Part model, mm, in its own coordinate system. Round coordinates to 2 decimals unless told otherwise and drop trailing zeros. Order: outer loops, then holes, each group sorted by start corner. A loop starts at its lowest first (then second) coordinate and runs counter-clockwise, first axis right, second up. Notation, with made-up numbers: (-7.75, -11) - (18.25, -11) arc R20 ccw to (18.25, 7) - close; hole circle Ø9 at (-30.75, -22.5). An arc over 180 degrees is marked (long way). Return JSON: item names as keys, results as strings. Group by question number.
Item 1: Drop flat-ended pins along their axis: pin 1 (6 mm diameter, centred on x = -35.5, y = -13.5, fed in from +Z); pin 2 (4 mm diameter, centred on y = 6.5, z = 427, fed in from +X); pin 3 (6 mm diameter, centred on x = 9.5, z = 217.5, fed in from -Y); pin 4 (1 mm diameter, centred on y = -16.5, z = 234, fed in from -X). Give the stop position or say it passes through.
Item 2: Probe probe 1 along Z at (x, y) = (0, -42); probe 2 along Y at (x, z) = (0, 487.5); probe 3 along X at (y, z) = (3, 461). List the from-to ranges inside material, lowest first.
Item 3: Two-plate mould, pull along Z, no slides. Class faces 1 (the face through (1.532, 42.374, 584.864)), 2 (the face through (-30.2, -26.5, 0)), 3 (the face through (-30.2, -26.5, 620)): released by +Z, released by -Z, zero draft, split by the parting line, or undercut.
Item 4: Saw through at C-C on x = 34. List the corners of the cut face in (y, z).
Item 5: Saw through at A-A on x = 0. List the corners of the cut face in (y, z), and give its area (3 significant figures).
Item 6: Saw through at B-B on y = 0. List the corners of the cut face in (x, z), and give its area (3 significant figures).
Item 7: Saw through at D-D on z = 351. List the corners of the cut face in (x, y), and give its area (3 significant figures).
```python
from build123d import *

# Parameters (mm, degrees)
SKETCH_1_R          = 45
SKETCH_1_R_2        = 40
EXTRUDE_1_DEPTH     = 40
SKETCH_2_R          = 50
SKETCH_2_R_2        = 40
EXTRUDE_2_DEPTH     = 30
SKETCH_3_R          = 45
SKETCH_3_R_2        = 40
EXTRUDE_3_DEPTH     = 550
SKETCH_4_R          = 5.1
CUT_EXTRUDE_1_DEPTH = 91
SKETCH_5_R          = 50
SKETCH_5_R_2        = 45
CUT_EXTRUDE_2_DEPTH = 117


with BuildPart() as part:
    # 草图1 → 凸台-拉伸1 (new body)
    with BuildSketch(Plane.XY):
        Circle(SKETCH_1_R)
        Circle(SKETCH_1_R_2, mode=Mode.SUBTRACT)
    extrude(amount=EXTRUDE_1_DEPTH)

    # 草图2 → 凸台-拉伸2 (add)
    with BuildSketch(Plane.XY.offset(40)):
        Circle(SKETCH_2_R)
        Circle(SKETCH_2_R_2, mode=Mode.SUBTRACT)
    extrude(amount=EXTRUDE_2_DEPTH)

    # 草图3 → 凸台-拉伸3 (add)
    with BuildSketch(Plane.XY.offset(70)):
        Circle(SKETCH_3_R)
        Circle(SKETCH_3_R_2, mode=Mode.SUBTRACT)
    extrude(amount=EXTRUDE_3_DEPTH)

    # 草图4 → 切除-拉伸1 (cut, symmetric)
    with BuildSketch(Plane(origin=(0, 0, 0), x_dir=(1, 0, 0), z_dir=(0, 1, 0))):
        with Locations(Location((0, -605, 0), (0, 0, 270))):
            Circle(SKETCH_4_R)
        with Locations(Location((0, -580, 0), (0, 0, 270))):
            Circle(SKETCH_4_R)
    extrude(amount=CUT_EXTRUDE_1_DEPTH, both=True, mode=Mode.SUBTRACT)

    # 草图5 → 切除-拉伸2 (cut)
    with BuildSketch(Plane(origin=(0, 0, 40), x_dir=(-1, 0, 0), z_dir=(0, 0, -1))):
        Circle(SKETCH_5_R)
        with Locations(Location((0, 0, 0), (0, 0, 180))):
            Circle(SKETCH_5_R_2, mode=Mode.SUBTRACT)
    extrude(amount=-CUT_EXTRUDE_2_DEPTH, mode=Mode.SUBTRACT)


solid = part.part
```
Filled in:
{
 "1": {"pin 1": "stops at z = 620", "pin 2": "stops at x = 44.77", "pin 3": "stops at y = -44.53", "pin 4": "stops at x = -42.06"},
 "2": {"probe 1": "z = 0 to 574.9, 585.1 to 599.9, 610.1 to 620", "probe 2": "y = -45 to -40, 40 to 45", "probe 3": "x = -44.9 to -39.89, 39.89 to 44.9"},
 "3": {"face 1": "undercut", "face 2": "released by -Z", "face 3": "released by +Z"},
 "4": {"outline": "(-29.48, 0) - (-21.07, 0) - (-21.07, 620) - (-29.48, 620) - close; (21.07, 0) - (29.48, 0) - (29.48, 620) - (21.07, 620) - close"},
 "5": {"outline": "(-45, 0) - (-40, 0) - (-40, 574.9) - (-45, 574.9) - close; (-45, 585.1) - (-40, 585.1) - (-40, 599.9) - (-45, 599.9) - close; (-45, 610.1) - (-40, 610.1) - (-40, 620) - (-45, 620) - close; (40, 0) - (45, 0) - (45, 574.9) - (40, 574.9) - close; (40, 585.1) - (45, 585.1) - (45, 599.9) - (40, 599.9) - close; (40, 610.1) - (45, 610.1) - (45, 620) - (40, 620) - close", "area": "6,000 mm^2"},
 "6": {"outline": "(-45, 0) - (-40, 0) - (-40, 620) - (-45, 620) - close; (40, 0) - (45, 0) - (45, 620) - (40, 620) - close", "area": "6,200 mm^2"},
 "7": {"outline": "circle Ø90 at (0, 0); hole circle Ø80 at (0, 0)", "area": "1,340 mm^2"}
}
